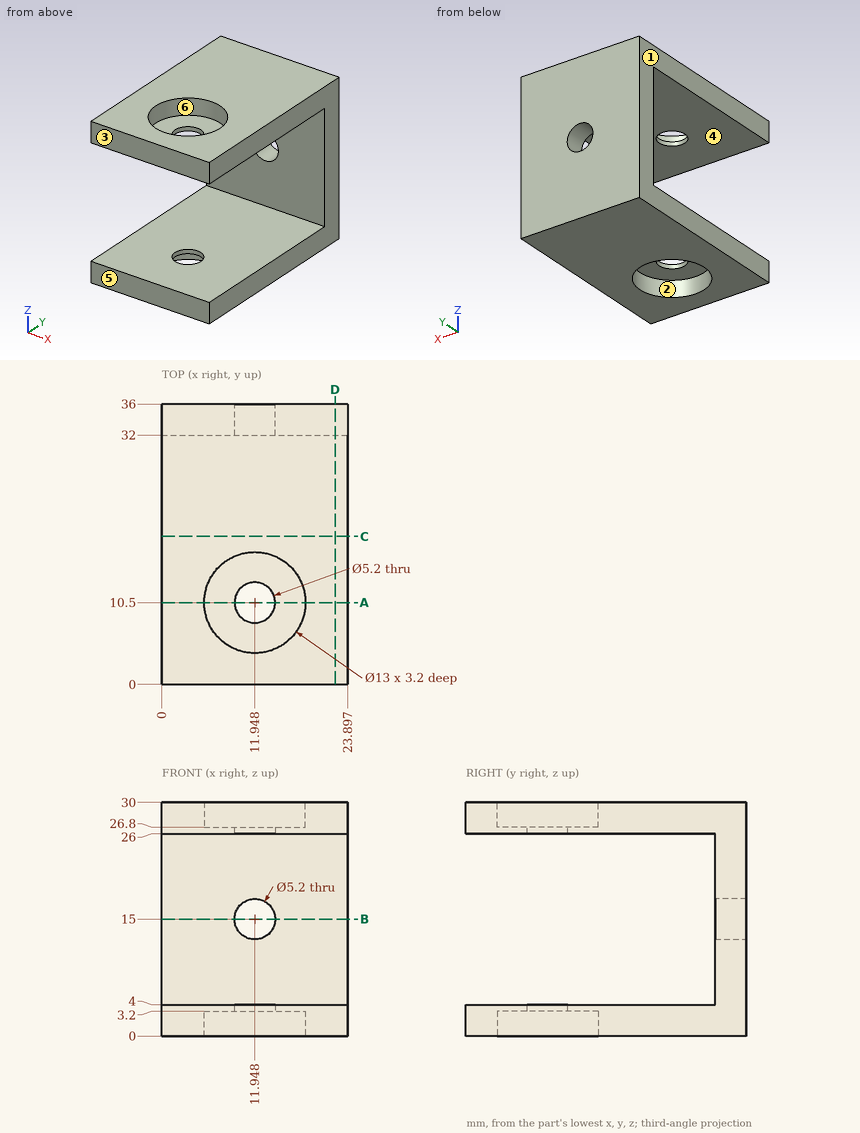
Part print with two shaded views. Sizes in mm from the minimum x, y, z corner. A direction names the side the tool comes from. Round coordinates to 2 decimals unless told otherwise and drop trailing zeros. Write each loop counter-clockwise with the first axis right and the second up, starting at its lowest first coordinate (ties: lowest second). Pieces come first, ordered by that corner, then holes. Notation, with made-up numbers: M 47.5,59 L 62.5,59 A27 cw 62.5,79 Z; hole C 50.5,-24 d6. An arc over 180 degrees is marked long. Put each result on its own line as item: value. Start each with the question number.
1) Drill centre lines: probe 1 along Z at (x, y) = (2.25, 18.5); probe 2 along Z at (x, y) = (11, 16); probe 3 along Y at (x, z) = (14.25, 18.5). Where is each one in solid material? Low to high. Write a range as [from, to].
2) Saw through at D-D, the plane x = 22.25. Write the cut outline in (y, z), and give its area (3 significant figures).
3) Saw through at C-C, the plane y = 19. Write the cut outline in (x, z).
4) Saw through at B-B, the plane z = 15. Write the cut outline in (x, y).
5) Pull direction Y, two halves, no side cores. Call the marked faces 1, 2 and 3: pulls with the +Y half, pulls with the -Y half, needs draft (parallel to the pull), parting line crosses it, or undercut.
6) Pin check, flat tips, straight feed: pin 1 Ø1.5 at (x, y) = (4, 22) entering from -Z; pin 2 Ø8 at (x, y) = (11.95, 10.5) entering from +Z; pin 3 Ø6 at (x, y) = (11.95, 10.5) entering from -Z; pin 4 Ø8 at (x, z) = (12.5, 14) entering from -Y. Stop position of each tip, or through.
7) Saw through at A-A, the plane y = 10.5. Write the cut outline in (x, z).
8) 3-axis set-ups, long thin cutter, end or side, ignore diameter. For the marked faces 4, 5 and 6: which of +Z, -Z, +X, -X, +Y, -Y reach the whole face in a straight line?
Resolved:
1. probe 1: [0, 4], [26, 30]
1. probe 2: [3.2, 4], [26, 26.8]
1. probe 3: [32, 36]
2. outline: M 0,0 L 36,0 L 36,30 L 0,30 L 0,26 L 32,26 L 32,4 L 0,4 Z
2. area: 376 mm²
3. outline: M 0,0 L 23.9,0 L 23.9,4 L 0,4 Z; M 0,26 L 23.9,26 L 23.9,30 L 0,30 Z
4. outline: M 0,32 L 9.35,32 L 9.35,36 L 0,36 Z; M 14.55,32 L 23.9,32 L 23.9,36 L 14.55,36 Z
5. face 1: needs draft
5. face 2: undercut
5. face 3: pulls with the -Y half
6. pin 1: z = 0
6. pin 2: z = 26.8
6. pin 3: z = 3.2
6. pin 4: y = 32
7. outline: M 0,0 L 5.45,0 L 5.45,3.2 L 9.35,3.2 L 9.35,4 L 0,4 Z; M 0,26 L 9.35,26 L 9.35,26.8 L 5.45,26.8 L 5.45,30 L 0,30 Z; M 14.55,3.2 L 18.45,3.2 L 18.45,0 L 23.9,0 L 23.9,4 L 14.55,4 Z; M 14.55,26 L 23.9,26 L 23.9,30 L 18.45,30 L 18.45,26.8 L 14.55,26.8 Z
8. face 4: +X, -X, -Y
8. face 5: +Z, -Z, +X, -X, -Y
8. face 6: +Z
